Job drawing, mm, ordinate dimensions from the low corner. One solid piece. Give positions to 0.01 mm unless a question says otherwise; leave off trailing zeros. Write each loop counter-clockwise with the first axis right and the second up, starting at its lowest first coordinate (ties: lowest second). Pieces come first, ordered by that corner, then holes. Notation, with made-up numbers: M -32.75,72.5 L -1.75,72.5 A12 cw -1.75,91.5 Z; hole C 85.5,-8.75 d6. An arc over 180 degrees is marked long. Answer as CSV lines item,"result". Start each with the question number.
1) Slice it at B-B, the plane x = 26. Give the cut face in (y, z).
2) Pin check, flat tip, straight feed: pin 1 Ø6.5 at (x, y) = (37.5, 68) entering from -Z. Stop position of the tip, or through.
3) Slice it at C-C, the plane y = 51. Give the cut face in (x, z), plus the area to 3 significant figures.
4) Slice it at A-A, the plane y = 37.5. Give the cut face in (x, z).
5) Wall check: line 1 along Y through (x, z) = (37.5, 0.45); line 2 along X through (y, z) = (20.5, 0.2); line 3 along X through (y, z) = (27, 0.15). Give the ranges that are in metal, low to high. Write a range as from..to.
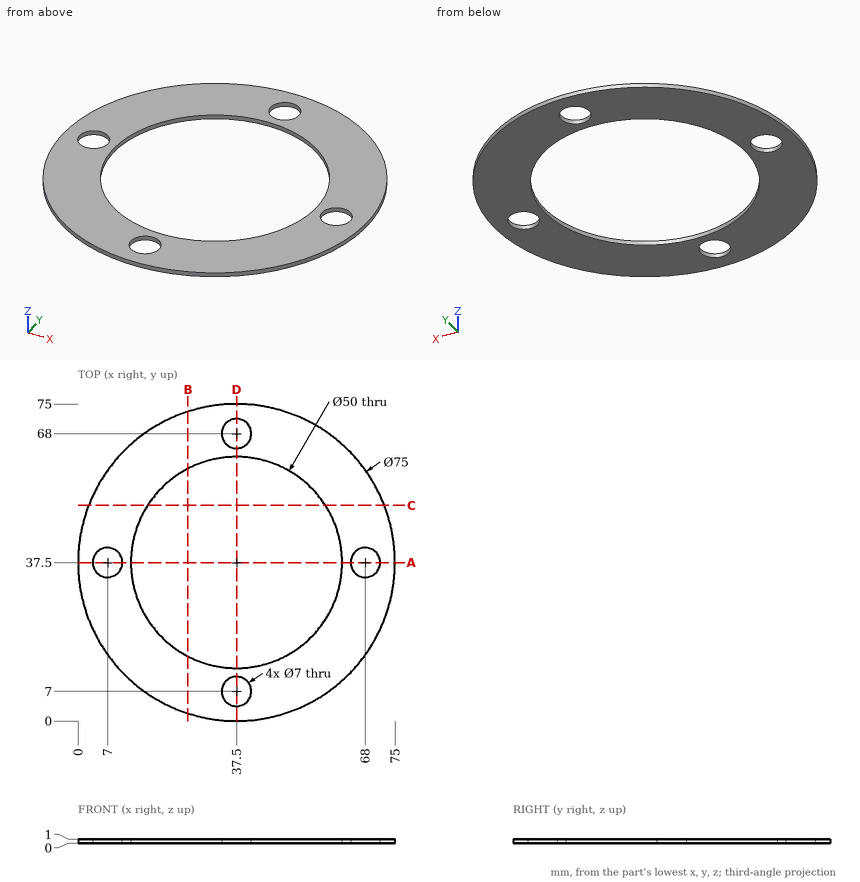
Found:
1,outline,"M 1.81,0 L 15.3,0 L 15.3,1 L 1.81,1 Z; M 59.7,0 L 73.19,0 L 73.19,1 L 59.7,1 Z"
2,pin 1,"through"
3,outline,"M 2.51,0 L 16.46,0 L 16.46,1 L 2.51,1 Z; M 58.54,0 L 72.49,0 L 72.49,1 L 58.54,1 Z"
3,area,"27.9 mm²"
4,outline,"M 0,0 L 3.5,0 L 3.5,1 L 0,1 Z; M 10.5,0 L 12.5,0 L 12.5,1 L 10.5,1 Z; M 62.5,0 L 64.5,0 L 64.5,1 L 62.5,1 Z; M 71.5,0 L 75,0 L 75,1 L 71.5,1 Z"
5,line 1,"0..3.5, 10.5..12.5, 62.5..64.5, 71.5..75"
5,line 2,"4.07..19.17, 55.83..70.93"
5,line 3,"1.5..14.81, 60.19..73.5"
